```python
from build123d import *

# Parameters (mm, degrees)
SKETCH_1_W              = 250
SKETCH_1_H              = 170
EXTRUDE_1_DEPTH         = 5
SKETCH_2_W              = 80
SKETCH_2_H              = 40
CUT_EXTRUDE_1_DEPTH     = 10
HOLE_WIZARD_9_0_9_1_D   = 9
PATTERN_LINEAR_1_COUNT  = 3
PATTERN_LINEAR_1_PITCH  = 110
HOLE_WIZARD_12_0_12_1_D = 12
SKETCH_7_R              = 15
CUT_EXTRUDE_2_DEPTH     = 10
HOLE_WIZARD_M6_1_D      = 5
FILLET_1_R              = 10


with BuildPart() as part:
    # 草图1 → 凸台-拉伸1 (new, symmetric)
    with BuildSketch(Plane.XY):
        Rectangle(SKETCH_1_W, SKETCH_1_H)
    extrude(amount=EXTRUDE_1_DEPTH, both=True)

    # 草图2 → 切除-拉伸1 (cut)
    with BuildSketch(Plane.XY.offset(5)):
        with Locations((85, 65)):
            Rectangle(SKETCH_2_W, SKETCH_2_H)
    cut_extrude_1 = extrude(amount=-CUT_EXTRUDE_1_DEPTH, mode=Mode.SUBTRACT)

    # 镜向1: 切除-拉伸1 across plane
    add(cut_extrude_1.mirror(Plane(origin=(0, 0, 0), x_dir=(0, 0, 1), z_dir=(1, 0, 0))), mode=Mode.SUBTRACT)

    # Ø9.0 (9) 直径孔1 (through all)
    with Locations(Plane.XY.offset(5)):
        with Locations((-110, -30), (-110, -70)):
            hole_wizard_9_0_9_1 = Hole(HOLE_WIZARD_9_0_9_1_D / 2)

    # 阵列(线性)1: Ø9.0 (9) 直径孔1 ×3
    with Locations(*[(i * PATTERN_LINEAR_1_PITCH, 0, 0) for i in range(1, PATTERN_LINEAR_1_COUNT)]):
        add(hole_wizard_9_0_9_1, mode=Mode.SUBTRACT)

    # Ø12.0 (12) 直径孔1 (through all)
    with Locations(Plane.XY.offset(5)):
        with Locations((-100, 35), (100, 35)):
            Hole(HOLE_WIZARD_12_0_12_1_D / 2)

    # 草图7 → 切除-拉伸2 (cut)
    with BuildSketch(Plane.XY.offset(5)):
        with Locations((0, 35)):
            Circle(SKETCH_7_R)
    extrude(amount=-CUT_EXTRUDE_2_DEPTH, mode=Mode.SUBTRACT)

    # M6 螺纹孔1 (through all)
    with Locations(Plane.XY.offset(5)):
        with Locations((-19.8, 15.2), (19.8, 54.8)):
            Hole(HOLE_WIZARD_M6_1_D / 2)

    # 圆角1
    fillet_1_edges = [part.edges().sort_by_distance(p)[0] for p in [
        (45, 85, 0),
        (125, 45, 0),
        (-45, 85, 0),
        (-125, 45, 0),
        (125, -85, 0),
        (-125, -85, 0),
    ]]
    fillet(fillet_1_edges, radius=FILLET_1_R)


solid = part.part
```
Source: CAD feature listing. Evaluate the final solid. Frame: model axes, mm. Coordinates: 2 decimals unless noted, no trailing zeros. Loops run counter-clockwise (first coordinate to the right, second up) from the corner with the lowest first, then second, coordinate; pieces in that order, holes last. Notation, with made-up numbers: M 75,64 L 110,64 A29 cw 110,86 Z; hole C 84.5,-15.75 d1. An arc over 180 degrees is marked long. Put each result on its own line as item: value. Start each with the question number.
1) Cut plane A-A on x = -19.8. Return the cut outline in (y, z).
2) Pull-direction query (Y, two-part tool) for faces 1 (the face through (-45, 60, 0)), 2 (the face through (-42.15, 81.99, -0.07)), 3 (the face through (-19.26, 12.76, -0.07)), 4 (the face through (-2, -85, 0)); classes: pulls with the +Y half, pulls with the -Y half, needs draft (parallel to the pull), parting line crosses it, or undercut.
3) Cut plane D-D on z = -3.5. Give the number of separate pieces and of enclosed holes in the cut face, then the cut area to 3 significant figures.
4) Cut plane B-B on y = 54.8. Return the cut outline in (x, z).
5) Contact query for flat-ended pins moving along their axis: pin 1 Ø12 at (x, y) = (-83.5, 47) entering from +Z; pin 2 Ø5 at (x, z) = (-91, -1.5) entering from +Y; pin 3 Ø5 at (y, z) = (58, 2) entering from +X; pin 4 Ø5 at (y, z) = (55.5, 2) entering from -X. Output: stop coordinate, or through.
6) Ray query, L1, parallel to Y at x = 110, z = -2.5; L2, parallel to Y at x = 0, z = -2.25; L3, parallel to Y at x = 3.5, z = 2.5. Return the intervals inside material, ascending. Write a range as from..to.
7) Cut plane C-C on x = 110. Return the cut outline in (y, z), then the cut area to 3 significant figures.
The answers:
1. outline: M -85,-5 L 12.7,-5 L 12.7,5 L -85,5 Z; M 17.7,-5 L 85,-5 L 85,5 L 17.7,5 Z
2. face 1: needs draft
2. face 2: pulls with the +Y half
2. face 3: undercut
2. face 4: pulls with the -Y half
3. separate pieces: 1
3. enclosed holes: 11
3. area: 34,600 mm²
4. outline: M -45,-5 L 17.3,-5 L 17.3,5 L -45,5 Z; M 22.3,-5 L 45,-5 L 45,5 L 22.3,5 Z
5. pin 1: stops at z = 5
5. pin 2: stops at y = 45
5. pin 3: stops at x = 45
5. pin 4: stops at x = -45
6. L1: y = -85..-74.5, -65.5..-34.5, -25.5..45
6. L2: y = -85..-74.5, -65.5..-34.5, -25.5..20, 50..85
6. L3: y = -85..-72.83, -67.17..-32.83, -27.17..20.41, 49.59..85
7. outline: M -85,-5 L -74.5,-5 L -74.5,5 L -85,5 Z; M -65.5,-5 L -34.5,-5 L -34.5,5 L -65.5,5 Z; M -25.5,-5 L 45,-5 L 45,5 L -25.5,5 Z
7. area: 1,120 mm²
